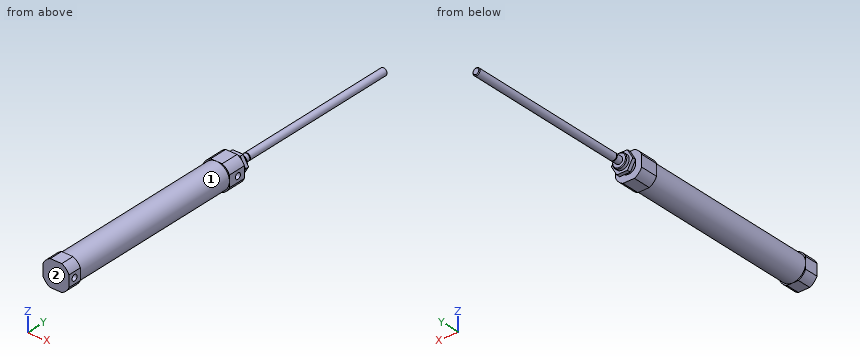
from build123d import *

# Parameters (mm, degrees)
BOSS_EXTRUDE1_DEPTH   = 12.5
SKETCH3_R             = 9.15
BOSS_EXTRUDE2_DEPTH   = 125
BOSS_EXTRUDE3_START   = 9.5
BOSS_EXTRUDE3_DEPTH   = 9.5
SKETCH5_R             = 5
BOSS_EXTRUDE4_DEPTH   = 8
SKETCH6_R             = 2.5
BOSS_EXTRUDE5_DEPTH   = 5
CHAMFER1_SIZE         = 0.5
SKETCH8_R             = 2.5
BOSS_EXTRUDE6_DEPTH   = 115
CHAMFER2_SIZE         = 0.5
BOSS_EXTRUDE7_DEPTH   = 2.5
CHAMFER4_SIZE         = 0.5
M5_TAPPED_HOLE1_D     = 4.2
M5_TAPPED_HOLE1_DEPTH = 14
M5_TAPPED_HOLE1_TIP   = 1.2618073


with BuildPart() as part:
    # Sketch1 → Boss-Extrude1 (new body)
    with BuildSketch(Plane(origin=(0, 0, 0), x_dir=(1, 0, 0), z_dir=(0, 1, 0))):
        with BuildLine():
            Line((-4.034538387, 9.15), (4.034538387, 9.15))
            ThreePointArc((4.034538387, 9.15), (7.071067812, 7.071067812), (9.15, 4.034538387))
            Line((9.15, 4.034538387), (9.15, -4.034538387))
            ThreePointArc((9.15, -4.034538387), (7.071067812, -7.071067812), (4.034538387, -9.15))
            Line((4.034538387, -9.15), (-4.034538387, -9.15))
            ThreePointArc((-4.034538387, -9.15), (-7.071067812, -7.071067812), (-9.15, -4.034538387))
            Line((-9.15, -4.034538387), (-9.15, 4.034538387))
            ThreePointArc((-9.15, 4.034538387), (-7.071067812, 7.071067812), (-4.034538387, 9.15))
        make_face()
    extrude(amount=BOSS_EXTRUDE1_DEPTH)

    # Sketch3 → Boss-Extrude2 (add)
    with BuildSketch(Plane.XZ):
        with Locations(Location((0, 0, 0), (0, 0, 270))):
            Circle(SKETCH3_R)
    extrude(amount=BOSS_EXTRUDE2_DEPTH)

    # Sketch4 → Boss-Extrude3 (add)
    with BuildSketch(Plane.XZ.offset(125).offset(BOSS_EXTRUDE3_START)):
        with BuildLine():
            Line((-4.034538387, 9.15), (4.034538387, 9.15))
            ThreePointArc((4.034538387, 9.15), (7.071067812, 7.071067812), (9.15, 4.034538387))
            Line((9.15, 4.034538387), (9.15, -4.034538387))
            ThreePointArc((9.15, -4.034538387), (7.071067812, -7.071067812), (4.034538387, -9.15))
            Line((4.034538387, -9.15), (-4.034538387, -9.15))
            ThreePointArc((-4.034538387, -9.15), (-7.071067812, -7.071067812), (-9.15, -4.034538387))
            Line((-9.15, -4.034538387), (-9.15, 4.034538387))
            ThreePointArc((-9.15, 4.034538387), (-7.071067812, 7.071067812), (-4.034538387, 9.15))
        make_face()
    extrude(amount=-BOSS_EXTRUDE3_DEPTH)

    # Sketch5 → Boss-Extrude4 (add)
    with BuildSketch(Plane(origin=(0, 12.5, 0), x_dir=(1, 0, 0), z_dir=(0, 1, 0))):
        with Locations(Location((0, 0, 0), (0, 0, 270))):
            Circle(SKETCH5_R)
    extrude(amount=BOSS_EXTRUDE4_DEPTH)

    # Sketch6 → Boss-Extrude5 (add)
    with BuildSketch(Plane(origin=(0, 20.5, 0), x_dir=(1, 0, 0), z_dir=(0, 1, 0))):
        with Locations(Location((0, 0, 0), (0, 0, 270))):
            Circle(SKETCH6_R)
    extrude(amount=BOSS_EXTRUDE5_DEPTH)

    # Chamfer1
    chamfer1_edges = [part.edges().sort_by_distance(p)[0] for p in [
        (0, 25.5, -2.5),
    ]]
    chamfer(chamfer1_edges, length=CHAMFER1_SIZE)

    # Sketch8 → Boss-Extrude6 (add)
    with BuildSketch(Plane(origin=(0, 25.5, 0), x_dir=(1, 0, 0), z_dir=(0, 1, 0))):
        with Locations(Location((0, 0, 0), (0, 0, 270))):
            Circle(SKETCH8_R)
    extrude(amount=BOSS_EXTRUDE6_DEPTH)

    # Chamfer2
    chamfer2_edges = [part.edges().sort_by_distance(p)[0] for p in [
        (0, 20.5, -5),
    ]]
    chamfer(chamfer2_edges, length=CHAMFER2_SIZE)

    # Sketch9 → Boss-Extrude7 (add)
    with BuildSketch(Plane(origin=(0, 15.5, 0), x_dir=(1, 0, 0), z_dir=(0, 1, 0))):
        Polygon((7.505553499, 0), (3.75277675, 6.5), (-3.75277675, 6.5), (-7.505553499, 0), (-3.75277675, -6.5), (3.75277675, -6.5), align=None)
    extrude(amount=BOSS_EXTRUDE7_DEPTH)

    # Chamfer4
    chamfer4_edges = [part.edges().sort_by_distance(p)[0] for p in [
        (0, 140.5, -2.5),
    ]]
    chamfer(chamfer4_edges, length=CHAMFER4_SIZE)

    # M5 Tapped Hole1
    with Locations(Plane(origin=(9.15, 0, 0), x_dir=(0, 0, -1), z_dir=(1, 0, 0))):
        with Locations((0, 7.109181896), (0, -129.804166053)):
            Hole(M5_TAPPED_HOLE1_D / 2, depth=M5_TAPPED_HOLE1_DEPTH)
            with Locations((0, 0, -(M5_TAPPED_HOLE1_DEPTH + M5_TAPPED_HOLE1_TIP / 2))):  # 118° drill point
                Cone(0, M5_TAPPED_HOLE1_D / 2, M5_TAPPED_HOLE1_TIP, mode=Mode.SUBTRACT)


solid = part.part
Geometry: final body of the model. Coordinates: model frame, mm. Face numbers are marked on the shaded views. Give positions to 0.01 mm unless a question says otherwise; leave off trailing zeros. Write each loop counter-clockwise with the first axis right and the second up, starting at its lowest first coordinate (ties: lowest second). Pieces come first, ordered by that corner, then holes. Notation, with made-up numbers: (-12, 32) -> (31, 32) arc R19 ccw to (31, 56) -> close; hole circle Ø3 at (27.25, 58.25). An arc over 180 degrees is marked (long way). Answer in a Markdown table with one row per item.
(1) Draft query along Y for the marked faces 1 and 2. Return one class per face: +Y half, -Y half, draft (parallel to the pull), parting line (faces both ways), or undercut.
Answers below:
| item | result |
|---|---|
| face 1 | undercut |
| face 2 | -Y half |
(2) Ray query, line 1 along Y through (x, z) = (6, 0); line 2 along Y through (x, z) = (-3, 0); line 3 along Y through (x, z) = (1.5, 0.75). Return the intervals inside material, ascending. Write a range as [from, to].
Answers below:
| item | result |
|---|---|
| line 1 | [-134.5, -131.9], [-127.7, 5.01], [9.21, 12.5], [15.5, 18] |
| line 2 | [-134.5, -131.9], [-127.7, 5.01], [9.21, 20.5] |
| line 3 | [-134.5, -131.77], [-127.84, 5.15], [9.07, 140.5] |
(3) Section query A-A on y = -29. Return loops of the section in (x, z).
Answers below:
| item | result |
|---|---|
| outline | circle Ø18.3 at (0, 0) |
(4) Section query B-B on y = 36.5. Return loops of the section in (x, z).
Answers below:
| item | result |
|---|---|
| outline | circle Ø5 at (0, 0) |
(5) Pin query (flat end, axial travel): pin 1 (3 mm diameter, centred on y = -35.5, z = 5.5, fed in from +X); pin 2 (1 mm diameter, centred on x = 3.5, z = -3, fed in from +Y); pin 3 (8 mm diameter, centred on y = -73, z = 7, fed in from +X); pin 4 (3 mm diameter, centred on y = 33, z = -5.5, fed in from +X). Return the tip coordinate at first contact, or that it passes through.
Answers below:
| item | result |
|---|---|
| pin 1 | x = 8.23 |
| pin 2 | y = 20.5 |
| pin 3 | x = 8.64 |
| pin 4 | through |
